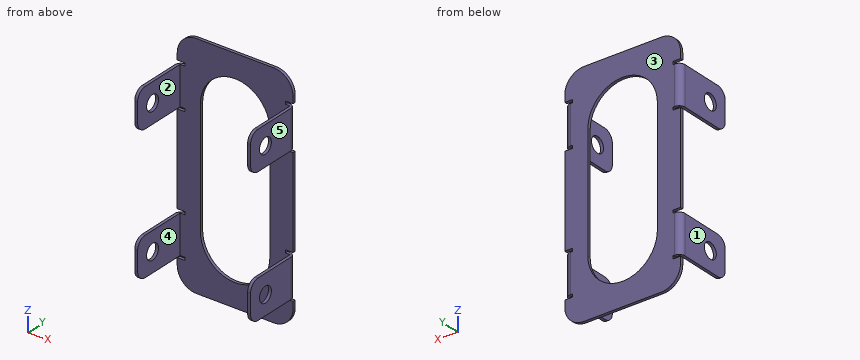
from build123d import *

# Parameters (mm, degrees)
COVER_PLATE_1_5MM_DEPTH    = 1.5
SIDE_A_LEGS_SKETCH_R       = 4
SIDE_A_MOUNTING_LEGS_DEPTH = 1.5
SIDE_START                 = -1.5
SIDE_B_LEGS_SKETCH_R       = 4
SIDE_B_MOUNTING_LEGS_DEPTH = 1.5
CORNER_FILLETS_R3_R        = 3
OBLONG_SLOT_CUT_DEPTH      = 1.5


with BuildPart() as part:
    # Cover Plate Sketch → Cover Plate 1.5mm (new body)
    with BuildSketch(Plane(origin=(0, 0, 0), x_dir=(1, 0, 0), z_dir=(0, 1, 0))):
        with BuildLine():
            Line((-30, 45), (-26, 45))
            Line((-26, 45), (-26, 46.5))
            Line((-26, 46.5), (-30, 46.5))
            Line((-30, 46.5), (-30, 50))
            ThreePointArc((-30, 50), (-27.071067812, 57.071067812), (-20, 60))
            Line((-20, 60), (20, 60))
            ThreePointArc((20, 60), (27.071067812, 57.071067812), (30, 50))
            Line((30, 50), (30, 46.5))
            Line((30, 46.5), (26, 46.5))
            Line((26, 46.5), (26, 45))
            Line((26, 45), (30, 45))
            Line((30, 45), (30, 25))
            Line((30, 25), (26, 25))
            Line((26, 25), (26, 23.5))
            Line((26, 23.5), (30, 23.5))
            Line((30, 23.5), (30, -23.5))
            Line((30, -23.5), (26, -23.5))
            Line((26, -23.5), (26, -25))
            Line((26, -25), (30, -25))
            Line((30, -25), (30, -45))
            Line((30, -45), (26, -45))
            Line((26, -45), (26, -46.5))
            Line((26, -46.5), (30, -46.5))
            Line((30, -46.5), (30, -50))
            ThreePointArc((30, -50), (27.071067812, -57.071067812), (20, -60))
            Line((20, -60), (-20, -60))
            ThreePointArc((-20, -60), (-27.071067812, -57.071067812), (-30, -50))
            Line((-30, -50), (-30, -46.5))
            Line((-30, -46.5), (-26, -46.5))
            Line((-26, -46.5), (-26, -45))
            Line((-26, -45), (-30, -45))
            Line((-30, -45), (-30, -25))
            Line((-30, -25), (-26, -25))
            Line((-26, -25), (-26, -23.5))
            Line((-26, -23.5), (-30, -23.5))
            Line((-30, -23.5), (-30, 23.5))
            Line((-30, 23.5), (-26, 23.5))
            Line((-26, 23.5), (-26, 25))
            Line((-26, 25), (-30, 25))
            Line((-30, 25), (-30, 45))
        make_face()
    extrude(amount=COVER_PLATE_1_5MM_DEPTH)

    # Side A Legs Sketch → Side A Mounting Legs (add)
    # profile 1 of 2: a face of its own
    with BuildSketch(Plane(origin=(30, 0, 0), x_dir=(0, 0, -1), z_dir=(1, 0, 0))):
        with BuildLine():
            Line((-45, 1.5), (-25, 1.5))
            Line((-25, 1.5), (-25, -23.5))
            ThreePointArc((-25, -23.5), (-26.464466094, -27.035533906), (-30, -28.5))
            Line((-30, -28.5), (-40, -28.5))
            ThreePointArc((-40, -28.5), (-43.535533906, -27.035533906), (-45, -23.5))
            Line((-45, -23.5), (-45, 1.5))
        make_face()
        with Locations((-35, -18.5)):
            Circle(SIDE_A_LEGS_SKETCH_R, mode=Mode.SUBTRACT)
    # profile 2 of 2: a face of its own
    with BuildSketch(Plane(origin=(30, 0, 0), x_dir=(0, 0, -1), z_dir=(1, 0, 0))):
        with BuildLine():
            Line((25, 1.5), (45, 1.5))
            Line((45, 1.5), (45, -23.5))
            ThreePointArc((45, -23.5), (43.535533906, -27.035533906), (40, -28.5))
            Line((40, -28.5), (30, -28.5))
            ThreePointArc((30, -28.5), (26.464466094, -27.035533906), (25, -23.5))
            Line((25, -23.5), (25, 1.5))
        make_face()
        with Locations((35, -18.5)):
            Circle(SIDE_A_LEGS_SKETCH_R, mode=Mode.SUBTRACT)
    extrude(amount=-SIDE_A_MOUNTING_LEGS_DEPTH)

    # Side B Legs Sketch → Side B Mounting Legs (add)
    # profile 1 of 2: a face of its own
    with BuildSketch(Plane.ZY.offset(30).offset(SIDE_START)):
        with BuildLine():
            Line((-45, 1.5), (-25, 1.5))
            Line((-25, 1.5), (-25, -23.5))
            ThreePointArc((-25, -23.5), (-26.464466094, -27.035533906), (-30, -28.5))
            Line((-30, -28.5), (-40, -28.5))
            ThreePointArc((-40, -28.5), (-43.535533906, -27.035533906), (-45, -23.5))
            Line((-45, -23.5), (-45, 1.5))
        make_face()
        with Locations(Location((-35, -18.5, 0), (0, 0, 180))):
            Circle(SIDE_B_LEGS_SKETCH_R, mode=Mode.SUBTRACT)
    # profile 2 of 2: a face of its own
    with BuildSketch(Plane.ZY.offset(30).offset(SIDE_START)):
        with BuildLine():
            Line((25, 1.5), (45, 1.5))
            Line((45, 1.5), (45, -23.5))
            ThreePointArc((45, -23.5), (43.535533906, -27.035533906), (40, -28.5))
            Line((40, -28.5), (30, -28.5))
            ThreePointArc((30, -28.5), (26.464466094, -27.035533906), (25, -23.5))
            Line((25, -23.5), (25, 1.5))
        make_face()
        with Locations(Location((35, -18.5, 0), (0, 0, 180))):
            Circle(SIDE_B_LEGS_SKETCH_R, mode=Mode.SUBTRACT)
    extrude(amount=SIDE_B_MOUNTING_LEGS_DEPTH)

    # Corner Fillets R3
    corner_fillets_r3_edges = [part.edges().sort_by_distance(p)[0] for p in [
        (-30, 1.5, -35),
        (-30, 1.5, 35),
        (30, 1.5, 35),
        (30, 1.5, -35),
    ]]
    fillet(corner_fillets_r3_edges, radius=CORNER_FILLETS_R3_R)

    # Oblong Slot Sketch → Oblong Slot Cut (cut)
    with BuildSketch(Plane(origin=(0, 1.5, 0), x_dir=(1, 0, 0), z_dir=(0, 1, 0))):
        with BuildLine():
            Line((-18, -30), (-18, 30))
            ThreePointArc((-18, 30), (0, 48), (18, 30))
            Line((18, 30), (18, -30))
            ThreePointArc((18, -30), (0, -48), (-18, -30))
        make_face()
    extrude(amount=-OBLONG_SLOT_CUT_DEPTH, mode=Mode.SUBTRACT)


solid = part.part
Can you work these out from the model? Positions are in its coordinate system, mm. Face numbers are marked on the shaded views. A direction names the side the tool comes from. Give positions to 0.01 mm unless a question says otherwise; leave off trailing zeros. Loops run counter-clockwise (first coordinate to the right, second up) from the corner with the lowest first, then second, coordinate; pieces in that order, holes last. Notation, with made-up numbers: (76, -9.75) -> (81, -9.75) arc R21 ccw to (81, -0.75) -> close; hole circle Ø7 at (-32.75, 32.5). An arc over 180 degrees is marked (long way). Write item = value, one per line.
1) Suppose I cut it at B-B on x = 0. Write out the boundary of the cut face in (y, z).
Check result:
outline = (0, -60) -> (1.5, -60) -> (1.5, -48) -> (0, -48) -> close; (0, 48) -> (1.5, 48) -> (1.5, 60) -> (0, 60) -> close
2) I need wall thicknesses on L1, parallel to X at y = -23, z = -30; L2, parallel to Y at x = -29.7, z = 35; L3, parallel to Y at x = -27, z = -33. Which ranges of each line are inside material? Lowest first, please. Write a range as from..to.
Check result:
L1 = -30..-28.5, 28.5..30
L2 = -28.5..-22.5, -14.5..-0.19
L3 = 0..1.5
3) For the marked faces 1 and 2, which set-ups out of +Z, -Z, +X, -X, +Y, -Y let a thin tool reach every point of the face, with its end or its side?
Check result:
face_1 = +Z, -Z, -X, +Y, -Y
face_2 = +Z, -Z, -Y
4) Suppose I cut it at A-A on y = -11. Write out the boundary of the cut face in (x, z).
Check result:
outline = (-30, -45) -> (-28.5, -45) -> (-28.5, -25) -> (-30, -25) -> close; (-30, 25) -> (-28.5, 25) -> (-28.5, 45) -> (-30, 45) -> close; (28.5, -45) -> (30, -45) -> (30, -25) -> (28.5, -25) -> close; (28.5, 25) -> (30, 25) -> (30, 45) -> (28.5, 45) -> close
5) Suppose I cut it at C-C on z = 4. Write out the boundary of the cut face in (x, y).
Check result:
outline = (-30, 0) -> (-18, 0) -> (-18, 1.5) -> (-30, 1.5) -> close; (18, 0) -> (30, 0) -> (30, 1.5) -> (18, 1.5) -> close
6) Thinking about a two-plate mould opening in X: for the marked faces 3, 4 and 5, which applies, released by +X, released by -X, zero draft, split by the parting line, or undercut?
Check result:
face_3 = zero draft
face_4 = undercut
face_5 = released by +X
7) Suppose I cut it at D-D on z = 36. Write out the boundary of the cut face in (x, y).
Check result:
outline = (-30, -28.5) -> (-28.5, -28.5) -> (-28.5, -22.37) -> (-30, -22.37) -> close; (-30, -14.63) -> (-28.5, -14.63) -> (-28.5, 0) -> (-16.97, 0) -> (-16.97, 1.5) -> (-27, 1.5) arc R3 ccw to (-30, -1.5) -> close; (16.97, 0) -> (28.5, 0) -> (28.5, -14.63) -> (30, -14.63) -> (30, -1.5) arc R3 ccw to (27, 1.5) -> (16.97, 1.5) -> close; (28.5, -28.5) -> (30, -28.5) -> (30, -22.37) -> (28.5, -22.37) -> close
8) Will these pins go through, and if not, where does the flat tip stop? pin 1 (1.2 mm diameter, centred on x = 28, y = -13, fed in from -Z); pin 2 (3 mm diameter, centred on x = 28, y = -12.5, fed in from +Z); pin 3 (0.8 mm diameter, centred on y = 1, z = -24, fed in from -X).
Check result:
pin_1 = -45
pin_2 = 45
pin_3 = -26
